from build123d import *

# Parameters (mm, degrees)
BASE_PLATE_DEPTH            = 290
MOUNTING_HOLES_SKETCH_R     = 7.5
MOUNTING_HOLES_10X_15_DEPTH = 290


with BuildPart() as part:
    # Plate Profile Sketch → Base Plate (new, symmetric)
    with BuildSketch(Plane.XY):
        Polygon((-124, 0), (-69, 0), (-69, -10), (69, -10), (69, 0), (124, 0), (124, 30), (-124, 30), align=None)
    extrude(amount=BASE_PLATE_DEPTH, both=True)

    # Mounting Holes Sketch → Mounting Holes 10xØ15 (cut, symmetric)
    with BuildSketch(Plane(origin=(0, 30, 0), x_dir=(1, 0, 0), z_dir=(0, 1, 0))):
        with Locations(Location((-92, 265, 0), (0, 0, 180))):
            Circle(MOUNTING_HOLES_SKETCH_R)
        with Locations(Location((-92, 132.5, 0), (0, 0, 180))):
            Circle(MOUNTING_HOLES_SKETCH_R)
        with Locations(Location((-92, 0, 0), (0, 0, 180))):
            Circle(MOUNTING_HOLES_SKETCH_R)
        with Locations(Location((-92, -132.5, 0), (0, 0, 180))):
            Circle(MOUNTING_HOLES_SKETCH_R)
        with Locations(Location((-92, -265, 0), (0, 0, 180))):
            Circle(MOUNTING_HOLES_SKETCH_R)
        with Locations(Location((92, 132.5, 0), (0, 0, 270))):
            Circle(MOUNTING_HOLES_SKETCH_R)
        with Locations(Location((92, 0, 0), (0, 0, 270))):
            Circle(MOUNTING_HOLES_SKETCH_R)
        with Locations(Location((92, -132.5, 0), (0, 0, 270))):
            Circle(MOUNTING_HOLES_SKETCH_R)
        with Locations(Location((92, -265, 0), (0, 0, 270))):
            Circle(MOUNTING_HOLES_SKETCH_R)
        with Locations(Location((92, 265, 0), (0, 0, 270))):
            Circle(MOUNTING_HOLES_SKETCH_R)
    extrude(amount=MOUNTING_HOLES_10X_15_DEPTH, both=True, mode=Mode.SUBTRACT)


solid = part.part
Source: CAD feature listing. Evaluate the final solid. Frame: model axes, mm. A direction names the side the tool comes from. Give positions to 0.01 mm unless a question says otherwise; leave off trailing zeros. Write each loop counter-clockwise with the first axis right and the second up, starting at its lowest first coordinate (ties: lowest second). Pieces come first, ordered by that corner, then holes. Notation, with made-up numbers: (-37.5, 25) - (-12.5, 25) arc R27 cw to (-12.5, 54) - close; hole circle Ø6 at (13, 16.25). An arc over 180 degrees is marked (long way). Write item = value, one per line. Start each with the question number.
Q1. Cut plane B-B, the plane x = -92. Return loops of the section in (y, z).
Q2. Material intervals for probe 1 along Z at (x, y) = (-92, 9); probe 2 along X at (y, z) = (10, 132); probe 3 along Y at (x, z) = (-78, -161), sorted ascending.
Q3. Cut plane C-C, the plane z = -175. Return loops of the section in (x, y).
Q4. Cut plane A-A, the plane z = 0. Return loops of the section in (x, y).
Q5. Draft query along X for faces 1 (the flat face through (69, -5, 4)), 2 (the flat face through (2, 30, 4)), 3 (the cylindrical face through (-91.024, 15.21, -125.064)). Return one class per face: +X half, -X half, draft (parallel to the pull), parting line (faces both ways), or undercut.
Q6. Reachability of faces 4 (the cylindrical face through (-91.024, 15.21, 139.936)), 5 (the flat face through (-69, -5, 4)), 6 (the flat face through (102, 0, 4)) from +Z, -Z, +X, -X, +Y, -Y: full face, straight path, thin tool, end or side. Return the list, or none.
Q7. Pin query (flat end, axial travel): pin 1 Ø19.5 at (x, z) = (-92, 265) entering from +Y; pin 2 Ø13.5 at (x, z) = (-92, -132.5) entering from -Y; pin 3 Ø17 at (x, z) = (92, 265) entering from -Y; pin 4 Ø3 at (y, z) = (-7, -84.5) entering from +X. Return the tip coordinate at first contact, or that it passes through.
Computed values:
q1.outline = (0, -290) - (30, -290) - (30, -272.5) - (0, -272.5) - close; (0, -257.5) - (30, -257.5) - (30, -140) - (0, -140) - close; (0, -125) - (30, -125) - (30, -7.5) - (0, -7.5) - close; (0, 7.5) - (30, 7.5) - (30, 125) - (0, 125) - close; (0, 140) - (30, 140) - (30, 257.5) - (0, 257.5) - close; (0, 272.5) - (30, 272.5) - (30, 290) - (0, 290) - close
q2.probe_1 = -290 to -272.5, -257.5 to -140, -125 to -7.5, 7.5 to 125, 140 to 257.5, 272.5 to 290
q2.probe_2 = -124 to -99.48, -84.52 to 84.52, 99.48 to 124
q2.probe_3 = 0 to 30
q3.outline = (-124, 0) - (-69, 0) - (-69, -10) - (69, -10) - (69, 0) - (124, 0) - (124, 30) - (-124, 30) - close
q4.outline = (-124, 0) - (-99.5, 0) - (-99.5, 30) - (-124, 30) - close; (-84.5, 0) - (-69, 0) - (-69, -10) - (69, -10) - (69, 0) - (84.5, 0) - (84.5, 30) - (-84.5, 30) - close; (99.5, 0) - (124, 0) - (124, 30) - (99.5, 30) - close
q5.face_1 = +X half
q5.face_2 = draft
q5.face_3 = undercut
q6.face_4 = +Y, -Y
q6.face_5 = +Z, -Z, -X, -Y
q6.face_6 = +Z, -Z, +X, -Y
q7.pin_1 = 30
q7.pin_2 = through
q7.pin_3 = 0
q7.pin_4 = 69
